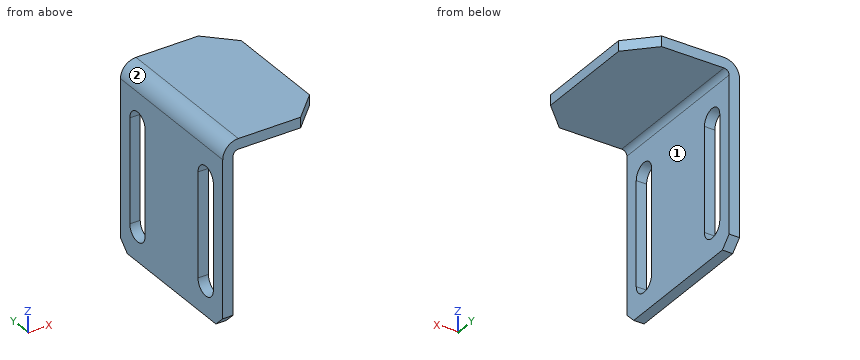
from build123d import *

# Parameters (mm, degrees)
BOSS_EXTRUDE1_DEPTH = 30
SKETCH3_R           = 2.25
CUT_EXTRUDE2_DEPTH  = 10
CHAMFER2_SIZE       = 2
FILLET1_R           = 1
FILLET2_R           = 3
CHAMFER3_SIZE       = 5
CUT_EXTRUDE3_DEPTH  = 10


with BuildPart() as part:
    # Sketch1 → Boss-Extrude1 (new body)
    with BuildSketch(Plane(origin=(0, 0, 0), x_dir=(1, 0, 0), z_dir=(0, 1, 0))):
        Polygon((0, 0), (20, 0), (20, 2), (2, 2), (2, 35), (0, 35), align=None)
    extrude(amount=BOSS_EXTRUDE1_DEPTH)

    # Sketch3 → Cut-Extrude2 (cut)
    with BuildSketch(Plane(origin=(2, 0, 0), x_dir=(0, 0, -1), z_dir=(1, 0, 0))):
        with Locations((29, 25)):
            Circle(SKETCH3_R)
        with Locations((29, 5)):
            Circle(SKETCH3_R)
    extrude(amount=-CUT_EXTRUDE2_DEPTH, mode=Mode.SUBTRACT)

    # Chamfer2
    chamfer2_edges = [part.edges().sort_by_distance(p)[0] for p in [
        (1, 30, -35),
        (1, 0, -35),
    ]]
    chamfer(chamfer2_edges, length=CHAMFER2_SIZE)

    # Fillet1
    fillet1_edges = [part.edges().sort_by_distance(p)[0] for p in [
        (2, 15, -2),
    ]]
    fillet(fillet1_edges, radius=FILLET1_R)

    # Fillet2
    fillet2_edges = [part.edges().sort_by_distance(p)[0] for p in [
        (0, 15, 0),
    ]]
    fillet(fillet2_edges, radius=FILLET2_R)

    # Chamfer3
    chamfer3_edges = [part.edges().sort_by_distance(p)[0] for p in [
        (20, 30, -1),
        (20, 0, -1),
    ]]
    chamfer(chamfer3_edges, length=CHAMFER3_SIZE)

    # Sketch4 → Cut-Extrude3 (cut)
    with BuildSketch(Plane(origin=(2, 0, 0), x_dir=(0, 0, -1), z_dir=(1, 0, 0))):
        with BuildLine():
            Line((29, 2.75), (9, 2.75))
            ThreePointArc((9, 2.75), (6.75, 5), (9, 7.25))
            Line((9, 7.25), (29, 7.25))
            ThreePointArc((29, 7.25), (31.25, 5), (29, 2.75))
        make_face()
        with BuildLine():
            Line((29, 27.25), (9, 27.25))
            ThreePointArc((9, 27.25), (6.75, 25), (9, 22.75))
            Line((9, 22.75), (29, 22.75))
            ThreePointArc((29, 22.75), (31.25, 25), (29, 27.25))
        make_face()
    extrude(amount=-CUT_EXTRUDE3_DEPTH, mode=Mode.SUBTRACT)


solid = part.part
Work out the finished part from the listing and answer in its coordinate system (mm). Face numbers are marked on the shaded views. A direction names the side the tool comes from. Coordinates: 2 decimals unless noted, no trailing zeros. Loops run counter-clockwise (first coordinate to the right, second up) from the corner with the lowest first, then second, coordinate; pieces in that order, holes last. Notation, with made-up numbers: M 24,64 L 81,64 A18 cw 81,85 Z; hole C 24,10 d7. An arc over 180 degrees is marked long. Answer in a Markdown table with one row per item. Add a question column.
1. Find section A-A, the plane z = -13.5. Write down the section's boundary in (x, y).
2. Find section D-D, the plane z = -7.5. Write down the section's boundary in (x, y).
3. Find section C-C, the plane x = 1. Write down the section's boundary in (y, z), then the cut area to 3 significant figures.
4. Flat-ended cylindrical pins translate along their axes: P1, Ø15, axis at y = 17.5, z = -22, coming from the +X side; P2, Ø10, axis at x = 17.5, y = 23, coming from the -Z side. Find the tip coordinate at first contact, or state that the pin passes through.
5. A tool of negligible diameter and unlimited length cuts with its end or side. For the marked faces 1 and 2, from which of +Z, -Z, +X, -X, +Y, -Y can it reach the whole face along a straight path? Write none if from no direction.
6. Consider L1, parallel to Z at x = 8.25, y = 3.5; L2, parallel to X at y = 11, z = -23.5; L3, parallel to Z at x = 1.5, y = 26.25. Determine where each line is inside the solid, lowest interval first.
7. Find section B-B, the plane y = 20.5. Write down the section's boundary in (x, z), then the cut area to 3 significant figures.
Reported:
| question | item | result |
|---|---|---|
| 1 | outline | M 0,0 L 2,0 L 2,2.75 L 0,2.75 Z; M 0,7.25 L 2,7.25 L 2,22.75 L 0,22.75 Z; M 0,27.25 L 2,27.25 L 2,30 L 0,30 Z |
| 2 | outline | M 0,0 L 2,0 L 2,3.32 L 0,3.32 Z; M 0,6.68 L 2,6.68 L 2,23.32 L 0,23.32 Z; M 0,26.68 L 2,26.68 L 2,30 L 0,30 Z |
| 3 | outline | M 0,-33 L 2,-35 L 28,-35 L 30,-33 L 30,-0.76 L 0,-0.76 Z; hole M 2.75,-29 A2.25 ccw 7.25,-29 L 7.25,-9 A2.25 ccw 2.75,-9 Z; hole M 22.75,-29 A2.25 ccw 27.25,-29 L 27.25,-9 A2.25 ccw 22.75,-9 Z |
| 3 | area | 811 mm^2 |
| 4 | P1 | stops at x = 2 |
| 4 | P2 | stops at z = -2 |
| 5 | face 1 | -Z, +X, +Y, -Y |
| 5 | face 2 | +Z, -X, +Y, -Y |
| 6 | L1 | z = -2 to 0 |
| 6 | L2 | x = 0 to 2 |
| 6 | L3 | z = -35 to -30.87, -7.13 to -0.4 |
| 7 | outline | M 0,-35 L 2,-35 L 2,-3 A1 cw 3,-2 L 20,-2 L 20,0 L 3,0 A3 ccw 0,-3 Z |
| 7 | area | 104 mm^2 |
